Verification items for the finished model (mm, model axes). Face numbers are marked on the shaded views. A direction names the side the tool comes from. Coordinates: 2 decimals unless noted, no trailing zeros. Write each loop counter-clockwise with the first axis right and the second up, starting at its lowest first coordinate (ties: lowest second). Pieces come first, ordered by that corner, then holes. Notation, with made-up numbers: (19.25, 70) -> (27.25, 70) arc R13 cw to (27.25, 85) -> close; hole circle Ø5 at (52, -30). An arc over 180 degrees is marked (long way). Use CSV: the item, a comma, the result in double quotes.
```python
from build123d import *

# Parameters (mm, degrees)
PLATE_BODY_12MM_DEPTH   = 12
THROUGH_HOLE_SKETCH_R   = 15
THROUGH_HOLE_DEPTH      = 12
FACE_POCKET_A_2MM_DEPTH = 2
FACE_POCKET_B_2MM_DEPTH = 2
SLOT_OPENING_CUT_DEPTH  = 10
RIM_NOTCH_A_SKETCH_W    = 6.711695518
RIM_NOTCH_A_SKETCH_H    = 52.229672595
RIM_NOTCH_A_DEPTH       = 10
RIM_NOTCH_B_SKETCH_W    = 2
RIM_NOTCH_B_SKETCH_H    = 52.229672595
RIM_NOTCH_B_DEPTH       = 10


with BuildPart() as part:
    # Plate Outline Sketch → Plate Body 12mm (new body)
    with BuildSketch(Plane.XY):
        with BuildLine():
            Line((0, -76), (0, 0))
            Line((0, 0), (0, 11.558252986))
            ThreePointArc((0, 11.558252986), (-10.446142685, 31.91035387), (-31.811209757, 40.087383673))
            ThreePointArc((-31.811209757, 40.087383673), (-41.331169578, 38.638494373), (-49.989043904, 34.423031486))
            ThreePointArc((-49.989043904, 34.423031486), (-87.99994879, -38.094936415), (-49.832664385, -110.530721493))
            ThreePointArc((-49.832664385, -110.530721493), (-41.198690561, -114.717276949), (-31.711695518, -116.155913677))
            ThreePointArc((-31.711695518, -116.155913677), (-10.653997006, -108.251003081), (0, -88.441747014))
            Line((0, -88.441747014), (0, -76))
        make_face()
    extrude(amount=PLATE_BODY_12MM_DEPTH)

    # Through Hole Sketch → Through Hole (cut)
    with BuildSketch(Plane.XY.offset(12)):
        with Locations((-62, -38.441747014)):
            Circle(THROUGH_HOLE_SKETCH_R)
    extrude(amount=-THROUGH_HOLE_DEPTH, mode=Mode.SUBTRACT)

    # Face Pocket A Sketch → Face Pocket A 2mm (cut)
    with BuildSketch(Plane.XY.offset(12)):
        with BuildLine():
            Line((-6.873473723, 8.080280991), (-6.899746136, -84.162980533))
            ThreePointArc((-6.899746136, -84.162980533), (-19.89556251, -105.973610229), (-45.263391889, -104.940148269))
            ThreePointArc((-45.263391889, -104.940148269), (-81.569163873, -38.072577616), (-45.50779291, 28.927113491))
            ThreePointArc((-45.50779291, 28.927113491), (-19.968976613, 30.033960698), (-6.873473723, 8.080280991))
        make_face()
    extrude(amount=-FACE_POCKET_A_2MM_DEPTH, mode=Mode.SUBTRACT)

    # Face Pocket B Sketch → Face Pocket B 2mm (cut)
    with BuildSketch(Plane(origin=(0, 0, 0), x_dir=(-1, 0, 0), z_dir=(0, 0, -1))):
        with BuildLine():
            Line((6.711695518, 8.087383673), (6.711695518, -84.155913677))
            ThreePointArc((6.711695518, -84.155913677), (19.751029382, -106.109101728), (45.267092765, -105.161893908))
            ThreePointArc((45.267092765, -105.161893908), (81.889710646, -38.07598005), (45.490730045, 29.131535823))
            ThreePointArc((45.490730045, 29.131535823), (19.839653868, 30.147924569), (6.711695518, 8.087383673))
        make_face()
    extrude(amount=-FACE_POCKET_B_2MM_DEPTH, mode=Mode.SUBTRACT)

    # Slot Opening Sketch → Slot Opening Cut (cut)
    with BuildSketch(Plane.XY.offset(10)):
        with BuildLine():
            Line((-12.997971015, -12.212074419), (-6.879253323, -12.212074419))
            Line((-6.879253323, -12.212074419), (0, -12.212074419))
            Line((0, -12.212074419), (0, -64.441747014))
            Line((0, -64.441747014), (-6.894129201, -64.441747014))
            Line((-6.894129201, -64.441747014), (-13.258551293, -64.441747014))
            ThreePointArc((-13.258551293, -64.441747014), (-28.540083812, -75.636809513), (-34.606755841, -57.691053721))
            ThreePointArc((-34.606755841, -57.691053721), (-28.520033449, -38.309557921), (-34.759611769, -18.976730106))
            ThreePointArc((-34.759611769, -18.976730106), (-28.558192424, -0.540946638), (-12.997971015, -12.212074419))
        make_face()
    extrude(amount=-SLOT_OPENING_CUT_DEPTH, mode=Mode.SUBTRACT)

    # Rim Notch A Sketch → Rim Notch A (cut)
    with BuildSketch(Plane(origin=(0, 0, 10), x_dir=(-1, 0, 0), z_dir=(0, 0, -1))):
        with Locations((3.355847759, -38.326910717)):
            Rectangle(RIM_NOTCH_A_SKETCH_W, RIM_NOTCH_A_SKETCH_H)
    extrude(amount=-RIM_NOTCH_A_DEPTH, mode=Mode.SUBTRACT)

    # Rim Notch B Sketch → Rim Notch B (cut)
    with BuildSketch(Plane(origin=(-6.711695518, 0, 0), x_dir=(0, 0, -1), z_dir=(1, 0, 0))):
        with Locations((-11, -38.326910717)):
            Rectangle(RIM_NOTCH_B_SKETCH_W, RIM_NOTCH_B_SKETCH_H)
    extrude(amount=-RIM_NOTCH_B_DEPTH, mode=Mode.SUBTRACT)


solid = part.part
```
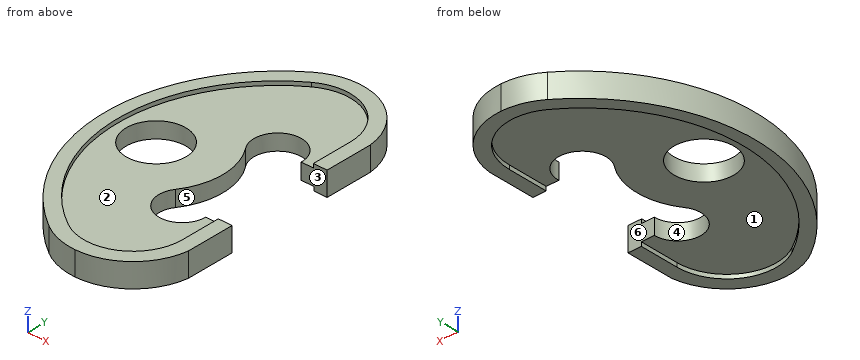
1) Cross-section at A-A (x = -60.5). Record the boundary of the cut face in (y, z), plus the area to 3 significant figures.
Return value:
outline,"(-101.9, 0) -> (-92.39, 0) -> (-92.39, 2) -> (-53.37, 2) -> (-53.37, 10) -> (-92.03, 10) -> (-92.03, 12) -> (-101.9, 12) -> close; (-23.52, 2) -> (16.51, 2) -> (16.51, 0) -> (25.9, 0) -> (25.9, 12) -> (16.18, 12) -> (16.18, 10) -> (-23.52, 10) -> close"
area,"861 mm2"
2) Cross-section at C-C (x = -30). Record the boundary of the cut face in (y, z), plus the area to 3 significant figures.
Return value:
outline,"(-116.11, 0) -> (-109.1, 0) -> (-109.1, 2) -> (-75.07, 2) -> (-75.07, 10) -> (-108.91, 10) -> (-108.91, 12) -> (-116.11, 12) -> close; (-48.29, 2) -> (-28.6, 2) -> (-28.6, 10) -> (-48.29, 10) -> close; (-1.09, 2) -> (33.12, 2) -> (33.12, 0) -> (40.04, 0) -> (40.04, 12) -> (32.96, 12) -> (32.96, 10) -> (-1.09, 10) -> close"
area,"871 mm2"
3) Cross-section at D-D (z = 5.75). Record the boundary of the cut face in (x, y).
Return value:
outline,"(-49.99, 34.42) arc R88 ccw to (-49.83, -110.53) arc R32 ccw to (0, -88.44) -> (0, -64.44) -> (-13.26, -64.44) arc R11.74 cw (long way) to (-34.61, -57.69) arc R33.48 ccw to (-34.76, -18.98) arc R12 cw (long way) to (-13, -12.21) -> (0, -12.21) -> (0, 11.56) arc R32 ccw to start; hole circle Ø30 at (-62, -38.44)"
4) Cross-section at B-B (y = -6.5). Record the boundary of the cut face in (x, z), plus the area to 3 significant figures.
Return value:
outline,"(-82.17, 0) -> (-75.45, 0) -> (-75.45, 2) -> (-35.66, 2) -> (-35.66, 10) -> (-75.14, 10) -> (-75.14, 12) -> (-82.17, 12) -> close; (-14.33, 2) -> (-6.71, 2) -> (-6.71, 0) -> (0, 0) -> (0, 12) -> (-6.88, 12) -> (-6.88, 10) -> (-14.33, 10) -> close"
area,"541 mm2"
5) Mould release check, pull along X, two halves, no side actions. Record for the marked faces 4, 5 and 6: released by +X, released by -X, zero draft, split by the parting line, or undercut.
Return value:
face 4,"undercut"
face 5,"released by +X"
face 6,"zero draft"
6) Set-up check for the marked faces 1, 2 and 3: record each of +Z, -Z, +X, -X, +Y, -Y from which the full face is reachable in a straight line by a thin tool's end or side.
Return value:
face 1,"-Z"
face 2,"+Z"
face 3,"+Z, -Z, +X"
7) Gauge pin test, flat ends, axial feed: pin 1 (1 mm diameter, centred on y = -73, z = 11, fed in from -X); pin 2 (1.6 mm diameter, centred on y = 3, z = 11, fed in from -X); pin 3 (3 mm diameter, centred on x = -49, z = 6.5, fed in from +Y); pin 4 (5 mm diameter, centred on y = 13, z = 1.5, fed in from +X). Record the tip position at first contact, or that the pin passes through.
Return value:
pin 1,"x = -80.96"
pin 2,"x = -78.28"
pin 3,"y = 35.98"
pin 4,"x = 0"
8) Scan lines: L1, parallel to Z at x = -44.5, y = -83; L2, parallel to Y at x = -56, z = 4; L3, parallel to Y at x = -31.5, z = 9.25. Record each from-to range of solid material in increasing order.
Return value:
L1,"2 to 10"
L2,"-105.88 to -52.19, -24.69 to 29.88"
L3,"-116.16 to -74.22, -52.25 to -24.63, -1.92 to 40.09"
